```python
from build123d import *

# Parameters (mm, degrees)
SKETCH_1_W                   = 115
SKETCH_1_H                   = 19
EXTRUDE_1_DEPTH              = 7.5
SKETCH_2_W                   = 72
SKETCH_2_H                   = 19
EXTRUDE_2_DEPTH              = 15
SKETCH_5_R                   = 23
CUT_EXTRUDE_3_DEPTH          = 6.5
CUT_EXTRUDE_START            = -9.2
SKETCH_6_R                   = 23
CUT_EXTRUDE_4_DEPTH          = 9.2
SKETCH_7_R                   = 21
CUT_EXTRUDE_5_DEPTH          = 63.998015842
FILLET_3_R                   = 2
CHAMFER_1_SIZE               = 0.5
SKETCH_8_W                   = 100
SKETCH_8_H                   = 30
CUT_EXTRUDE_8_DEPTH          = 3
SKETCH_12_W                  = 43
SKETCH_12_H                  = 3
CUT_EXTRUDE_9_DEPTH          = 61.178899957
SKETCH_13_W                  = 72
SKETCH_13_H                  = 13
CUT_EXTRUDE_10_DEPTH         = 64.099128362
SKETCH_14_W                  = 43
SKETCH_14_H                  = 15
EXTRUDE_3_DEPTH              = 16
SKETCH_16_W                  = 115
SKETCH_16_H                  = 3
CUT_EXTRUDE_14_DEPTH         = 64.784794426
CHAMFER_2_SIZE               = 10
HOLE_WIZARD_M5_1_D           = 5.5
HOLE_WIZARD_M5_1_CBORE_D     = 10
HOLE_WIZARD_M5_1_CBORE_DEPTH = 5.4
SKETCH_19_W                  = 25.462348227
SKETCH_19_H                  = 32.507755261
CUT_EXTRUDE_15_DEPTH         = 63.789330304


with BuildPart() as part:
    # 草图1 → 凸台-拉伸1 (new, symmetric)
    with BuildSketch(Plane(origin=(0, 0, 0), x_dir=(1, 0, 0), z_dir=(0, 1, 0))):
        Rectangle(SKETCH_1_W, SKETCH_1_H)
    extrude(amount=EXTRUDE_1_DEPTH, both=True)

    # 草图2 → 凸台-拉伸2 (add)
    with BuildSketch(Plane(origin=(0, 7.5, 0), x_dir=(1, 0, 0), z_dir=(0, 1, 0))):
        with Locations((-21.5, 0)):
            Rectangle(SKETCH_2_W, SKETCH_2_H)
    extrude(amount=EXTRUDE_2_DEPTH)

    # 草图5 → 切除-拉伸3 (cut)
    with BuildSketch(Plane.XY.offset(9.5)):
        with Locations((-32.5, 35)):
            Circle(SKETCH_5_R)
    extrude(amount=-CUT_EXTRUDE_3_DEPTH, mode=Mode.SUBTRACT)

    # 草图6 → 切除-拉伸4 (cut)
    with BuildSketch(Plane(origin=(0, 0, -9.5), x_dir=(-1, 0, 0), z_dir=(0, 0, -1)).offset(CUT_EXTRUDE_START)):
        with Locations((32.5, 35)):
            Circle(SKETCH_6_R)
    extrude(amount=CUT_EXTRUDE_4_DEPTH, mode=Mode.SUBTRACT)

    # 草图7 → 切除-拉伸5 (cut, through all)
    with BuildSketch(Plane.XY.offset(3)):
        with Locations((-32.5, 35)):
            Circle(SKETCH_7_R)
    extrude(amount=-CUT_EXTRUDE_5_DEPTH, mode=Mode.SUBTRACT)

    # 圆角3
    fillet_3_edges = [part.edges().sort_by_distance(p)[0] for p in [
        (-49.374537031, 22.5, 1.35),
        (-15.625462969, 22.5, 1.35),
    ]]
    fillet(fillet_3_edges, radius=FILLET_3_R)

    # 倒角1
    chamfer_1_edges = [part.edges().sort_by_distance(p)[0] for p in [
        (-51.080152824, 22.5, 3),
        (-13.919847176, 22.5, -0.3),
        (-32.5, 14, 3),
        (-32.5, 14, -0.3),
        (-51.080152824, 22.5, -0.3),
        (-49.493844118, 22.305787796, -0.3),
        (-15.506155882, 22.305787796, -0.3),
        (-13.919847176, 22.5, 3),
        (-49.493844118, 22.305787796, 3),
        (-15.506155882, 22.305787796, 3),
    ]]
    chamfer(chamfer_1_edges, length=CHAMFER_1_SIZE)

    # 草图8 → 切除-拉伸8 (cut)
    with BuildSketch(Plane.XY.offset(9.5)):
        with Locations((-35.5, 7.5)):
            Rectangle(SKETCH_8_W, SKETCH_8_H)
    cut_extrude_8 = extrude(amount=-CUT_EXTRUDE_8_DEPTH, mode=Mode.SUBTRACT)

    # 镜向1: 切除-拉伸8 across plane
    add(cut_extrude_8.mirror(Plane.XY), mode=Mode.SUBTRACT)

    # 草图12 → 切除-拉伸9 (cut, through all)
    with BuildSketch(Plane(origin=(0, 7.5, 0), x_dir=(1, 0, 0), z_dir=(0, 1, 0))):
        with Locations((36, 8)):
            Rectangle(SKETCH_12_W, SKETCH_12_H)
    extrude(amount=-CUT_EXTRUDE_9_DEPTH, mode=Mode.SUBTRACT)

    # 草图13 → 切除-拉伸10 (cut, through all)
    with BuildSketch(Plane.XY.offset(6.5)):
        with Locations((-21.5, -1)):
            Rectangle(SKETCH_13_W, SKETCH_13_H)
    extrude(amount=-CUT_EXTRUDE_10_DEPTH, mode=Mode.SUBTRACT)

    # 草图14 → 凸台-拉伸3 (add)
    with BuildSketch(Plane.XY.offset(9.5)):
        with Locations((36, 15)):
            Rectangle(SKETCH_14_W, SKETCH_14_H)
    extrude(amount=-EXTRUDE_3_DEPTH)

    # 草图16 → 切除-拉伸14 (cut, through all)
    with BuildSketch(Plane.XY.offset(9.5)):
        with Locations((0, 21)):
            Rectangle(SKETCH_16_W, SKETCH_16_H)
    extrude(amount=-CUT_EXTRUDE_14_DEPTH, mode=Mode.SUBTRACT)

    # 倒角2
    chamfer_2_edges = [part.edges().sort_by_distance(p)[0] for p in [
        (14.5, 5.5, 0),
    ]]
    chamfer(chamfer_2_edges, length=CHAMFER_2_SIZE)

    # M5 六角凹头螺钉的柱形沉头孔1 (through all)
    with Locations(Plane(origin=(0, 19.5, 0), x_dir=(1, 0, 0), z_dir=(0, 1, 0))):
        with Locations((23.5, -1.5), (48.5, -1.5)):
            CounterBoreHole(HOLE_WIZARD_M5_1_D / 2, HOLE_WIZARD_M5_1_CBORE_D / 2, HOLE_WIZARD_M5_1_CBORE_DEPTH)

    # 草图19 → 切除-拉伸15 (cut, through all)
    with BuildSketch(Plane(origin=(0, 0, -6.5), x_dir=(-1, 0, 0), z_dir=(0, 0, -1))):
        with Locations((52.231174114, 11.069476533)):
            Rectangle(SKETCH_19_W, SKETCH_19_H)
    extrude(amount=-CUT_EXTRUDE_15_DEPTH, mode=Mode.SUBTRACT)


solid = part.part
```
CAD build for the part. Positions are in the model's coordinates, mm. A direction names the side the tool comes from. Round coordinates to 2 decimals unless told otherwise and drop trailing zeros. Order: outer loops, then holes, each group sorted by start corner. A loop starts at its lowest first (then second) coordinate and runs counter-clockwise, first axis right, second up.
Item 1: Saw through at C-C on z = 1.5. Write the cut outline in (x, y).
Item 2: Saw through at D-D on y = 7. Write the cut outline in (x, z).
Item 3: Saw through at A-A on x = 23.5. Write the cut outline in (y, z).
Item 4: Mould opens along Z. For faces 1 (the face through (51, 14.1, 4)), 2 (the face through (36, 6, 9.5)), 3 (the face through (-28.48, 14.39, 1.37)), 4 (the face through (18.505, 16.838, 1.28)) say: pulls with the +Z half, pulls with the -Z half, needs draft (parallel to the pull), parting line crosses it, or undercut.
Item 5: Tool access for faces 5 (the face through (-18, 5.5, 0)), 6 (the face through (26, 14.1, 4)), 7 (the face through (-27, 14, -0.3)): list every direction of +Z, -Z, +X, -X, +Y, -Y with a clear straight run to the whole face (end or side of a thin tool).
Item 6: Saw through at B-B on y = 2.25. Write the cut outline in (x, z).
Item 7: Pin check, flat tips, straight feed: pin 1 (9 mm diameter, centred on x = 48.5, z = 1.5, fed in from +Y); pin 2 (2 mm diameter, centred on x = -29.5, y = 14, fed in from -Z); pin 3 (6.5 mm diameter, centred on x = -13, z = -3, fed in from -Y); pin 4 (3.5 mm diameter, centred on x = 23.5, z = 1.5, fed in from +Y). Stop position of each tip, or through.
Item 8: Probe line 1 along Z through (x, y) = (48.5, 8.75); line 2 along X through (y, z) = (10, 2.75); line 3 along Z through (x, y) = (13, 14.25). List the from-to ranges inside material, lowest first.
Reported:
1. outline: (-39.5, 5.5) - (4.5, 5.5) - (14.5, -4.5) - (14.5, -7.5) - (20.75, -7.5) - (20.75, 14.1) - (18.5, 14.1) - (18.5, 19.5) - (-18.33, 19.5) arc R21 cw to (-39.5, 15.2) - close; (26.25, -7.5) - (45.75, -7.5) - (45.75, 14.1) - (43.5, 14.1) - (43.5, 19.5) - (28.5, 19.5) - (28.5, 14.1) - (26.25, 14.1) - close; (51.25, -7.5) - (57.5, -7.5) - (57.5, 19.5) - (53.5, 19.5) - (53.5, 14.1) - (51.25, 14.1) - close
2. outline: (-39.5, -6.5) - (57.5, -6.5) - (57.5, 9.5) - (14.5, 9.5) - (14.5, 6.5) - (-39.5, 6.5) - close; hole circle Ø5.5 at (23.5, 1.5); hole circle Ø5.5 at (48.5, 1.5)
3. outline: (-7.5, -6.5) - (19.5, -6.5) - (19.5, -3.5) - (14.1, -3.5) - (14.1, -1.25) - (-7.5, -1.25) - close; (-7.5, 4.25) - (14.1, 4.25) - (14.1, 6.5) - (19.5, 6.5) - (19.5, 9.5) - (-7.5, 9.5) - close
4. face 1: undercut
4. face 2: pulls with the +Z half
4. face 3: needs draft
4. face 4: undercut
5. face 5: +Z, -Z, -X, -Y
5. face 6: +Y
5. face 7: -Z, +Y
6. outline: (7.75, -6.5) - (57.5, -6.5) - (57.5, 9.5) - (14.5, 9.5) - (14.5, 6.5) - (7.75, 6.5) - close; hole circle Ø5.5 at (23.5, 1.5); hole circle Ø5.5 at (48.5, 1.5)
7. pin 1: stops at y = 14.1
7. pin 2: stops at z = -0.3
7. pin 3: stops at y = 5.5
7. pin 4: passes through
8. line 1: z = -6.5 to -1.25, 4.25 to 9.5
8. line 2: x = -39.5 to 21.05, 25.95 to 46.05, 50.95 to 57.5
8. line 3: z = -6.5 to 6.5
